The model under review builds one solid part; all positions refer to its coordinate system, in mm. Face numbers are marked on the shaded views. A direction names the side the tool comes from. Give positions to 0.01 mm unless a question says otherwise; leave off trailing zeros. Order: outer loops, then holes, each group sorted by start corner. A loop starts at its lowest first (then second) coordinate and runs counter-clockwise, first axis right, second up. Notation, with made-up numbers: (5.5, 52) - (64.5, 52) arc R26 ccw to (64.5, 84) - close; hole circle Ø10 at (-17.75, 66). An arc over 180 degrees is marked (long way). Put each result on its own line as item: value.
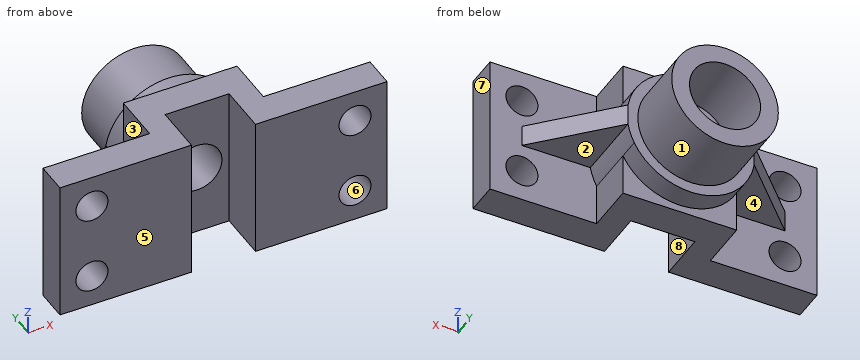
```python
from build123d import *

# Parameters (mm, degrees)
STEPPED_BASE_DEPTH          = 20
COLLAR_36_SKETCH_R          = 18
COLLAR_36_DEPTH             = 20
COLLAR_TRIM_SKETCH_W        = 18
COLLAR_TRIM_SKETCH_H        = 5
COLLAR_TRIM_CUT_DEPTH       = 68.505555327
HUB_30_SKETCH_R             = 15
HUB_30_DEPTH                = 18
COUNTERBORE_20_SKETCH_R     = 10
COUNTERBORE_20_DEPTH        = 18
BORE_14_SKETCH_R            = 7
BORE_14_DEPTH               = 58.939623747
MOUNTING_HOLE_9_SKETCH_R    = 4.5
MOUNTING_HOLES_9_DEPTH      = 63.92853089
SUPPORT_START               = -20
SUPPORT_RIB_DEPTH           = 20
RIB_TRIM_CUT_DEPTH          = 70.670653793
MIRRORED_RIB_TRIM_CUT_DEPTH = 70.670653793


with BuildPart() as part:
    # Base Profile Sketch → Stepped Base (new, symmetric)
    with BuildSketch(Plane.XY):
        Polygon((-46, 0), (-9, 0), (-9, 14), (9, 14), (9, 0), (46, 0), (46, 9), (16, 9), (16, 23), (-16, 23), (-16, 9), (-46, 9), align=None)
    extrude(amount=STEPPED_BASE_DEPTH, both=True)

    # Collar Ø36 Sketch → Collar Ø36 (add)
    with BuildSketch(Plane(origin=(0, 9, 0), x_dir=(1, 0, 0), z_dir=(0, 1, 0))):
        with Locations(Location((0, 0, 0), (0, 0, 27.266044451))):
            Circle(COLLAR_36_SKETCH_R)
    extrude(amount=COLLAR_36_DEPTH)

    # Collar Trim Sketch → Collar Trim Cut (cut, through all)
    with BuildSketch(Plane.XY.offset(20)):
        with Locations((0, 11.5)):
            Rectangle(COLLAR_TRIM_SKETCH_W, COLLAR_TRIM_SKETCH_H)
    extrude(amount=-COLLAR_TRIM_CUT_DEPTH, mode=Mode.SUBTRACT)

    # Hub Ø30 Sketch → Hub Ø30 (add)
    with BuildSketch(Plane(origin=(0, 29, 0), x_dir=(1, 0, 0), z_dir=(0, 1, 0))):
        with Locations(Location((0, 0, 0), (0, 0, 180))):
            Circle(HUB_30_SKETCH_R)
    extrude(amount=HUB_30_DEPTH)

    # Counterbore Ø20 Sketch → Counterbore Ø20 (cut)
    with BuildSketch(Plane(origin=(0, 47, 0), x_dir=(1, 0, 0), z_dir=(0, 1, 0))):
        with Locations(Location((0, 0, 0), (0, 0, 180))):
            Circle(COUNTERBORE_20_SKETCH_R)
    extrude(amount=-COUNTERBORE_20_DEPTH, mode=Mode.SUBTRACT)

    # Bore Ø14 Sketch → Bore Ø14 (cut, through all)
    with BuildSketch(Plane(origin=(0, 29, 0), x_dir=(1, 0, 0), z_dir=(0, 1, 0))):
        with Locations(Location((0, 0, 0), (0, 0, 180))):
            Circle(BORE_14_SKETCH_R)
    extrude(amount=-BORE_14_DEPTH, mode=Mode.SUBTRACT)

    # Mounting Hole Ø9 Sketch → Mounting Holes Ø9 (cut, through all)
    with BuildSketch(Plane(origin=(0, 9, 0), x_dir=(1, 0, 0), z_dir=(0, 1, 0))):
        with Locations(Location((37, -11, 0), (0, 0, 180))):
            Circle(MOUNTING_HOLE_9_SKETCH_R)
        with Locations(Location((37, 11, 0), (0, 0, 180))):
            Circle(MOUNTING_HOLE_9_SKETCH_R)
    mounting_holes_9 = extrude(amount=-MOUNTING_HOLES_9_DEPTH, mode=Mode.SUBTRACT)

    # Support Rib Sketch → Support Rib (add)
    with BuildSketch(Plane(origin=(0, 29, 0), x_dir=(1, 0, 0), z_dir=(0, 1, 0)).offset(SUPPORT_START)):
        with BuildLine():
            Line((37, 3), (37, -3))
            Line((37, -3), (17.748239349, -3))
            ThreePointArc((17.748239349, -3), (18, 0), (17.748239349, 3))
            Line((17.748239349, 3), (37, 3))
        make_face()
    support_rib = extrude(amount=SUPPORT_RIB_DEPTH)

    # Rib Trim Sketch → Rib Trim Cut (cut, through all)
    with BuildSketch(Plane.XY.offset(3)):
        Polygon((17.748239349, 29), (37, 9), (37, 29), align=None)
    extrude(amount=-RIB_TRIM_CUT_DEPTH, mode=Mode.SUBTRACT)

    # Rib and Holes Mirror: Mounting Holes Ø9, Support Rib across plane
    add(mounting_holes_9.mirror(Plane(origin=(0, 0, 0), x_dir=(0, 0, 1), z_dir=(1, 0, 0))), mode=Mode.SUBTRACT)
    add(support_rib.mirror(Plane(origin=(0, 0, 0), x_dir=(0, 0, 1), z_dir=(1, 0, 0))))

    # Mirrored Rib Trim Sketch → Mirrored Rib Trim Cut (cut, through all)
    with BuildSketch(Plane.XY.offset(3)):
        Polygon((-17.748239349, 29), (-37, 9), (-37, 29), align=None)
    extrude(amount=-MIRRORED_RIB_TRIM_CUT_DEPTH, mode=Mode.SUBTRACT)


solid = part.part
```
(1) The part is to be moulded in two halves that separate along X. For the marked faces 5, 6, 7 and 8, say which applies: pulls with the +X half, pulls with the -X half, needs draft (parallel to the pull), parting line crosses it, or undercut.
The answers:
face 5: needs draft
face 6: undercut
face 7: pulls with the +X half
face 8: undercut
(2) Wall thickness on L1, parallel to Z at x = -37, y = 6; L2, parallel to X at y = 5, z = -1; L3, parallel to Z at x = 0, y = 43.25: over which ranges is each line inside the solid? List them lowest first.
The answers:
L1: -20 to -15.5, -6.5 to 6.5, 15.5 to 20
L2: -46 to -9, 9 to 46
L3: -15 to -10, 10 to 15
(3) Take a section at D-D, the plane x = 23.5. Write out the cut boundary in (y, z), then the cut area to 3 significant figures.
The answers:
outline: (0, -20) - (9, -20) - (9, -3) - (23.02, -3) - (23.02, 3) - (9, 3) - (9, 20) - (0, 20) - close
area: 444 mm^2
(4) For the marked faces 1, 2, 3 and 4, list the 3-axis set-ups (+Z, -Z, +X, -X, +Y, -Y) from which the entire face can be reached by the end or side of a thin tool; tool diameter is ignored.
The answers:
face 1: +Y
face 2: -Z, +X, +Y
face 3: +Z, -X, +Y
face 4: -Z, -X, +Y
(5) Clearance check with flat-ended pins moving along their axes: pin 1 Ø7 at (x, z) = (37, 11) entering from +Y; pin 2 Ø15 at (x, z) = (28, 7) entering from +Y; pin 3 Ø6 at (y, z) = (17.5, 16) entering from +X; pin 4 Ø9.5 at (y, z) = (18.5, -12.5) entering from -X. State where each tip first meets the part, or that it passes through.
The answers:
pin 1: through
pin 2: y = 24.94
pin 3: x = 16
pin 4: x = -16.25
(6) Take a section at C-C, the plane z = -4. Write out the cut boundary in (x, y), then the cut area to 3 significant figures.
The answers:
outline: (-46, 0) - (-9, 0) - (-9, 14) - (-5.74, 14) - (-5.74, 29) - (-9.17, 29) - (-9.17, 47) - (-14.46, 47) - (-14.46, 29) - (-17.55, 29) - (-17.55, 9) - (-46, 9) - close; (5.74, 14) - (9, 14) - (9, 0) - (46, 0) - (46, 9) - (17.55, 9) - (17.55, 29) - (14.46, 29) - (14.46, 47) - (9.17, 47) - (9.17, 29) - (5.74, 29) - close
area: 1,300 mm^2
(7) Take a section at A-A, the plane x = 0. Write out the cut boundary in (y, z), then the cut area to 3 significant figures.
The answers:
outline: (14, -20) - (23, -20) - (23, -18) - (29, -18) - (29, -15) - (47, -15) - (47, -10) - (29, -10) - (29, -7) - (14, -7) - close; (14, 7) - (29, 7) - (29, 10) - (47, 10) - (47, 15) - (29, 15) - (29, 18) - (23, 18) - (23, 20) - (14, 20) - close
area: 546 mm^2
(8) Take a section at B-B, the plane y = 37. Write out the cut boundary in (x, z).
The answers:
outline: circle Ø30 at (0, 0); hole circle Ø20 at (0, 0)
